Here's how the part is built. I have some questions about the finished solid (model axes, mm). A direction names the side the tool comes from. Round coordinates to 2 decimals unless told otherwise and drop trailing zeros. Write each loop counter-clockwise with the first axis right and the second up, starting at its lowest first coordinate (ties: lowest second). Pieces come first, ordered by that corner, then holes. Notation, with made-up numbers: (37, 81) -> (47, 81) arc R8 ccw to (47, 92) -> close; hole circle Ø2 at (-10.75, 75). An arc over 180 degrees is marked (long way). Put each result on its own line as item: value. Start each with the question number.
1. Suppose I cut it at A-A (x = 5). Please give me the cut outline in (y, z).
2. Suppose I cut it at C-C (x = 19). Please give me the cut outline in (y, z).
3. Suppose I cut it at B-B (y = 37.5). Please give me the cut outline in (x, z).
4. Which directions (+Z, -Z, +X, -X, +Y, -Y) give clear straight access to the entire face, cutting with the end or side of a thin tool? Please do faces 4 (the face through (68.075, 38.183, 4.754)), 5 (the face through (10, 19, 2)), 6 (the face through (35, 22, 5)).
5. Suppose I cut it at D-D (z = 3.75). Please give me the cut outline in (x, y).
6. We'd pull the mould along X, two halves only. Please class faces 1 (the face through (35, 43, 2)), 2 (the face through (28, 19, 2)), 3 (the face through (0, 22, 2)): +X half, -X half, draft (parallel to the pull), parting line (faces both ways), or undercut.
7. I need wall thicknesses on probe 1 along Y at (x, z) = (65, 4.7); probe 2 along X at (y, z) = (17.5, 0.6); probe 3 along Y at (x, z) = (65, 0.75). Which ranges of each line are inside material? Lowest first, please. Write a range as from..to.
8. For pin 1 (8 mm diameter, centred on x = 17.5, y = 29.5, fed in from +Z); pin 2 (2 mm diameter, centred on x = 19, y = 27.5, fed in from +Z); pin 3 (4 mm diameter, centred on x = 5, y = 37.5, fed in from +Z); pin 4 (5 mm diameter, centred on x = 65, y = 37.5, fed in from +Z), each with a flat end and sliding along its axis, tell me the tip position at first contact or that it passes through.
```python
from build123d import *

# Parameters (mm, degrees)
BOSS_EXTRUDE1_DEPTH                            = 5
CSK_FOR_M3_FLAT_HEAD_MACHINE_SCREW1_AT_2_COUNT = 2
CSK_FOR_M3_FLAT_HEAD_MACHINE_SCREW1_AT_2_PITCH = 32
CSK_FOR_M3_FLAT_HEAD_MACHINE_SCREW1_AT_3_COUNT = 2
CSK_FOR_M3_FLAT_HEAD_MACHINE_SCREW1_AT_3_PITCH = 68
CSK_FOR_M3_FLAT_HEAD_MACHINE_SCREW1_AT_4_COUNT = 2
CSK_FOR_M3_FLAT_HEAD_MACHINE_SCREW1_AT_4_PITCH = 60


with BuildPart() as part:
    # Sketch1 → Boss-Extrude1 (new body)
    with BuildSketch(Plane.XY):
        with BuildLine():
            Line((2, 0), (68, 0))
            ThreePointArc((68, 0), (69.414213562, 0.585786438), (70, 2))
            Line((70, 2), (70, 41))
            ThreePointArc((70, 41), (69.414213562, 42.414213562), (68, 43))
            Line((68, 43), (2, 43))
            ThreePointArc((2, 43), (0.585786438, 42.414213562), (0, 41))
            Line((0, 41), (0, 2))
            ThreePointArc((0, 2), (0.585786438, 0.585786438), (2, 0))
        make_face()
        with BuildLine():
            Line((28, 21.5), (28, 16.5))
            ThreePointArc((28, 16.5), (19, 7.5), (10, 16.5))
            Line((10, 16.5), (10, 21.5))
            ThreePointArc((10, 21.5), (19, 30.5), (28, 21.5))
        make_face(mode=Mode.SUBTRACT)
        with BuildLine():
            Line((60, 21.5), (60, 16.5))
            ThreePointArc((60, 16.5), (51, 7.5), (42, 16.5))
            Line((42, 16.5), (42, 21.5))
            ThreePointArc((42, 21.5), (51, 30.5), (60, 21.5))
        make_face(mode=Mode.SUBTRACT)
    extrude(amount=BOSS_EXTRUDE1_DEPTH)

    # Sketch2 → CSK for M3 Flat Head Machine Screw1 (revolve, cut)
    with BuildSketch(Plane(origin=(5, 37.5, 5), x_dir=(0, -1, 0), z_dir=(1, 0, 0))):
        Polygon((0, 0), (0, 5), (1.6, 5), (1.6, 2.05), (3.15, 0.5), (3.15, 0), align=None)
    csk_for_m3_flat_head_machine_screw1 = revolve(axis=Axis((5, 37.5, 11.35), (0, 0, -1)), mode=Mode.SUBTRACT)

    # CSK for M3 Flat Head Machine Screw1 at 2: CSK for M3 Flat Head Machine Screw1 ×2
    with Locations(*[(0, -i * CSK_FOR_M3_FLAT_HEAD_MACHINE_SCREW1_AT_2_PITCH, 0) for i in range(1, CSK_FOR_M3_FLAT_HEAD_MACHINE_SCREW1_AT_2_COUNT)]):
        add(csk_for_m3_flat_head_machine_screw1, mode=Mode.SUBTRACT)

    # CSK for M3 Flat Head Machine Screw1 at 3: CSK for M3 Flat Head Machine Screw1 ×2
    with Locations(*[Vector(0.8823529411764707, -0.47058823529411764, 0) * (i * CSK_FOR_M3_FLAT_HEAD_MACHINE_SCREW1_AT_3_PITCH) for i in range(1, CSK_FOR_M3_FLAT_HEAD_MACHINE_SCREW1_AT_3_COUNT)]):
        add(csk_for_m3_flat_head_machine_screw1, mode=Mode.SUBTRACT)

    # CSK for M3 Flat Head Machine Screw1 at 4: CSK for M3 Flat Head Machine Screw1 ×2
    with Locations(*[(i * CSK_FOR_M3_FLAT_HEAD_MACHINE_SCREW1_AT_4_PITCH, 0, 0) for i in range(1, CSK_FOR_M3_FLAT_HEAD_MACHINE_SCREW1_AT_4_COUNT)]):
        add(csk_for_m3_flat_head_machine_screw1, mode=Mode.SUBTRACT)


solid = part.part
```
Verdict:
1. outline: (0, 0) -> (3.9, 0) -> (3.9, 2.95) -> (2.35, 4.5) -> (2.35, 5) -> (0, 5) -> close; (7.1, 0) -> (35.9, 0) -> (35.9, 2.95) -> (34.35, 4.5) -> (34.35, 5) -> (8.65, 5) -> (8.65, 4.5) -> (7.1, 2.95) -> close; (39.1, 0) -> (43, 0) -> (43, 5) -> (40.65, 5) -> (40.65, 4.5) -> (39.1, 2.95) -> close
2. outline: (0, 0) -> (7.5, 0) -> (7.5, 5) -> (0, 5) -> close; (30.5, 0) -> (43, 0) -> (43, 5) -> (30.5, 5) -> close
3. outline: (0, 0) -> (3.4, 0) -> (3.4, 2.95) -> (1.85, 4.5) -> (1.85, 5) -> (0, 5) -> close; (6.6, 0) -> (63.4, 0) -> (63.4, 2.95) -> (61.85, 4.5) -> (61.85, 5) -> (8.15, 5) -> (8.15, 4.5) -> (6.6, 2.95) -> close; (66.6, 0) -> (70, 0) -> (70, 5) -> (68.15, 5) -> (68.15, 4.5) -> (66.6, 2.95) -> close
4. face 4: +Z
4. face 5: +Z, -Z
4. face 6: +Z, +X, -X, +Y, -Y
5. outline: (0, 2) arc R2 ccw to (2, 0) -> (68, 0) arc R2 ccw to (70, 2) -> (70, 41) arc R2 ccw to (68, 43) -> (2, 43) arc R2 ccw to (0, 41) -> close; hole circle Ø4.8 at (5, 5.5); hole circle Ø4.8 at (5, 37.5); hole (10, 16.5) arc R9 ccw to (28, 16.5) -> (28, 21.5) arc R9 ccw to (10, 21.5) -> close; hole (42, 16.5) arc R9 ccw to (60, 16.5) -> (60, 21.5) arc R9 ccw to (42, 21.5) -> close; hole circle Ø4.8 at (65, 5.5); hole circle Ø4.8 at (65, 37.5)
6. face 1: draft
6. face 2: undercut
6. face 3: -X half
7. probe 1: y = 0..2.35, 8.65..34.35, 40.65..43
7. probe 2: x = 0..10, 28..42, 60..70
7. probe 3: y = 0..3.9, 7.1..35.9, 39.1..43
8. pin 1: stops at z = 5
8. pin 2: passes through
8. pin 3: stops at z = 3.35
8. pin 4: stops at z = 3.85
